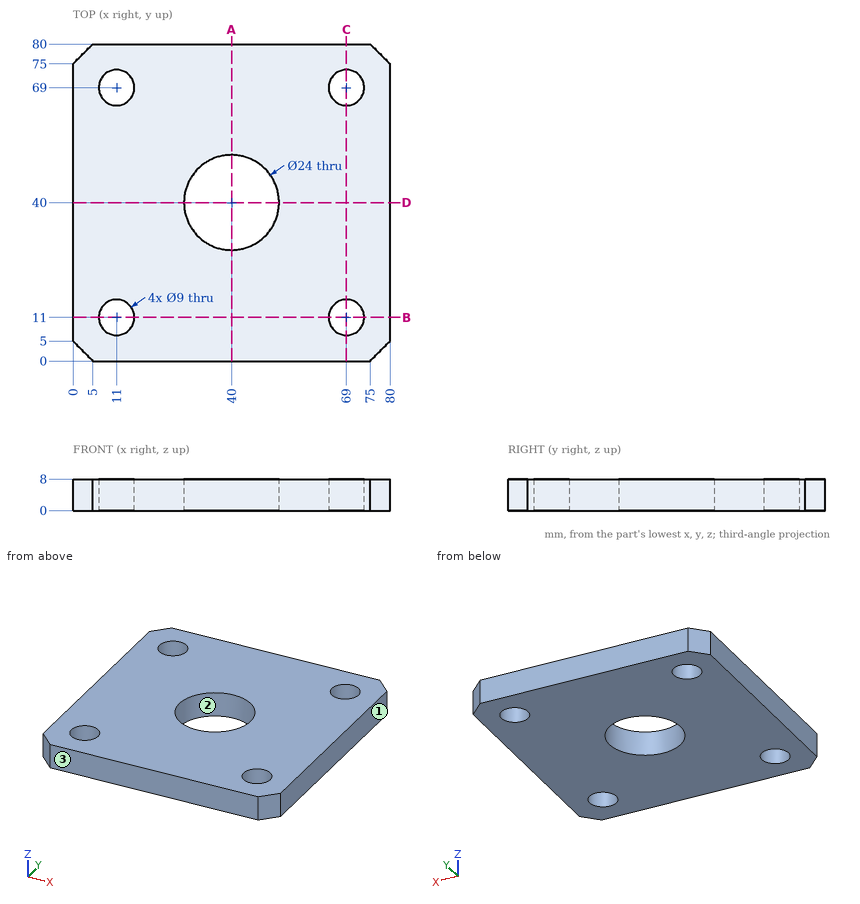
Can you work these out from the drawing? Everything is in mm from the part's minimum corner. Give positions to 0.01 mm unless a question says otherwise; leave off trailing zeros. Loops run counter-clockwise (first coordinate to the right, second up) from the corner with the lowest first, then second, coordinate; pieces in that order, holes last. Notation, with made-up numbers: (-36, 37) -> (-18, 37) arc R30 cw to (-18, 68) -> close; hole circle Ø1 at (27, 65). An arc over 180 degrees is marked (long way). Return JSON: item names as keys, results as strings.
Item 1: We'd pull the mould along Y, two halves only. Please class the marked faces 1, 2 and 3: +Y half, -Y half, draft (parallel to the pull), parting line (faces both ways), or undercut.
Geometry results:
{"face 1": "draft", "face 2": "undercut", "face 3": "-Y half"}
Item 2: I need wall thicknesses on L1, parallel to Y at x = 11, z = 4.75; L2, parallel to Y at x = 40, z = 6; L3, parallel to X at y = 10, z = 2.75. Which ranges of each line are inside material? Lowest first, please. Write a range as from..to.
Geometry results:
{"L1": "y = 0..6.5, 15.5..64.5, 73.5..80", "L2": "y = 0..28, 52..80", "L3": "x = 0..6.61, 15.39..64.61, 73.39..80"}
Item 3: If we section it at A-A on x = 40: List the corners of the cut face in (y, z) for me, plus the area to 3 significant figures.
Geometry results:
{"outline": "(0, 0) -> (28, 0) -> (28, 8) -> (0, 8) -> close; (52, 0) -> (80, 0) -> (80, 8) -> (52, 8) -> close", "area": "448 mm²"}
Item 4: If we section it at B-B on y = 11: List the corners of the cut face in (x, z) for me, plus the area to 3 significant figures.
Geometry results:
{"outline": "(0, 0) -> (6.5, 0) -> (6.5, 8) -> (0, 8) -> close; (15.5, 0) -> (64.5, 0) -> (64.5, 8) -> (15.5, 8) -> close; (73.5, 0) -> (80, 0) -> (80, 8) -> (73.5, 8) -> close", "area": "496 mm²"}
